Here's the drawing with two shaded views (mm, measured from the low corner). I have some questions. A direction names the side the tool comes from. Give positions to 0.01 mm unless a question says otherwise; leave off trailing zeros. Loops run counter-clockwise (first coordinate to the right, second up) from the corner with the lowest first, then second, coordinate; pieces in that order, holes last. Notation, with made-up numbers: (-18.75, 26) -> (29.25, 26) arc R17 cw to (29.25, 37) -> close; hole circle Ø8 at (57, 52.25). An arc over 180 degrees is marked (long way). Write each question's results on one line, items separated by ' | '. Start each with the question number.
Q1. Which directions (+Z, -Z, +X, -X, +Y, -Y) give clear straight access to the entire face, cutting with the end or side of a thin tool? Please do the marked faces 5, 6 and 7.
Q2. If we section it at D-D, the plane z = 5: List the corners of the cut face in (x, y) for me, plus the area to 3 significant figures.
Q3. If we section it at B-B, the plane z = 23.5: List the corners of the cut face in (x, y) for me.
Q4. If we section it at C-C, the plane y = 7: List the corners of the cut face in (x, z) for me.
Q5. If I drill on line 1 along X through (y, z) = (14, 5); line 2 along X through (y, z) = (1.25, 32); line 3 along X through (y, z) = (7.75, 16), over which ranges is the centre line in solid material (lowest first)?
Q6. Will these pins go through, and if not, where does the flat tip stop? P1, Ø16, axis at x = 81, z = 19.5, coming from the +Y side; P2, Ø5.5, axis at y = 8, z = 22.5, coming from the -X side; P3, Ø1.5, axis at y = 7.5, z = 18, coming from the +X side; P4, Ø2.5, axis at x = 27, z = 5, coming from the -Y side.
Q7. We'd pull the mould along X, two halves only. Please class the marked faces 1, 2, 3 and 4: released by +X, released by -X, zero draft, split by the parting line, or undercut.
Q8. If we section it at A-A, the plane x = 55.5: List the corners of the cut face in (y, z) for me.
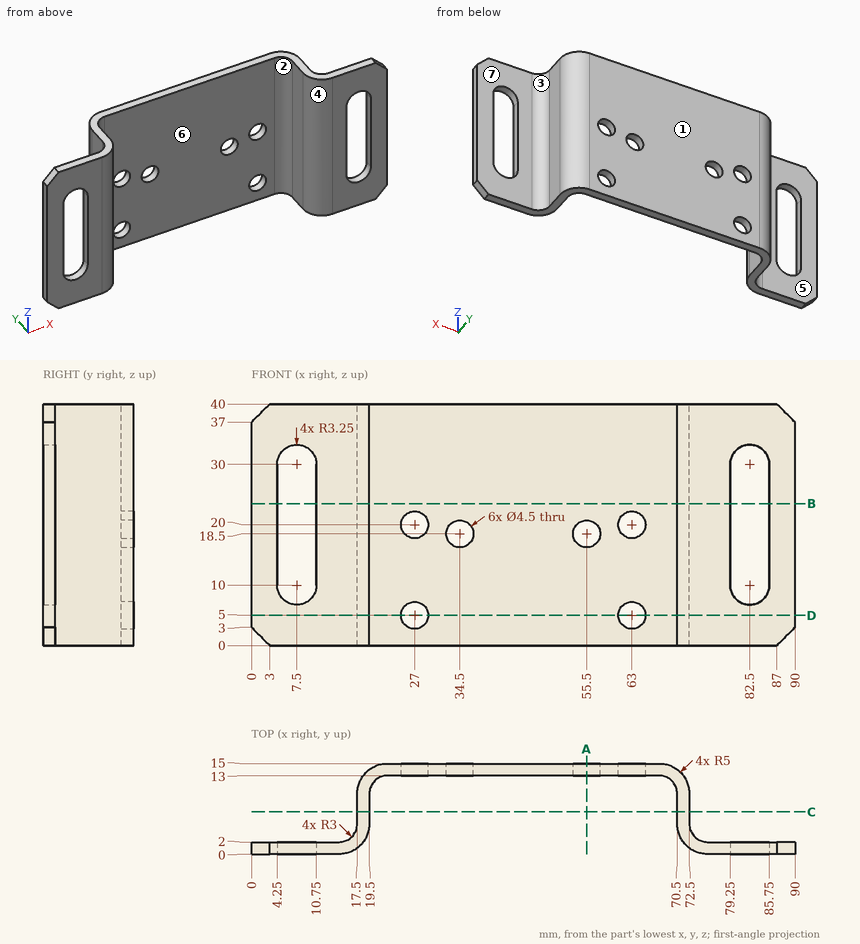
Final values:
1) face 5: +Z, -Z, -X, +Y | face 6: +Z, -Z, -Y | face 7: +Z, -Z, +X, +Y
2) outline: (0, 0) -> (14.5, 0) arc R5 ccw to (19.5, 5) -> (19.5, 10) arc R3 cw to (22.5, 13) -> (24.75, 13) -> (24.75, 15) -> (22.5, 15) arc R5 ccw to (17.5, 10) -> (17.5, 5) arc R3 cw to (14.5, 2) -> (0, 2) -> close; (29.25, 13) -> (60.75, 13) -> (60.75, 15) -> (29.25, 15) -> close; (65.25, 13) -> (67.5, 13) arc R3 cw to (70.5, 10) -> (70.5, 5) arc R5 ccw to (75.5, 0) -> (90, 0) -> (90, 2) -> (75.5, 2) arc R3 cw to (72.5, 5) -> (72.5, 10) arc R5 ccw to (67.5, 15) -> (65.25, 15) -> close | area: 200 mm²
3) outline: (0, 0) -> (4.25, 0) -> (4.25, 2) -> (0, 2) -> close; (10.75, 0) -> (14.5, 0) arc R5 ccw to (19.5, 5) -> (19.5, 10) arc R3 cw to (22.5, 13) -> (67.5, 13) arc R3 cw to (70.5, 10) -> (70.5, 5) arc R5 ccw to (75.5, 0) -> (79.25, 0) -> (79.25, 2) -> (75.5, 2) arc R3 cw to (72.5, 5) -> (72.5, 10) arc R5 ccw to (67.5, 15) -> (22.5, 15) arc R5 ccw to (17.5, 10) -> (17.5, 5) arc R3 cw to (14.5, 2) -> (10.75, 2) -> close; (85.75, 0) -> (90, 0) -> (90, 2) -> (85.75, 2) -> close
4) outline: (17.5, 0) -> (19.5, 0) -> (19.5, 40) -> (17.5, 40) -> close; (70.5, 0) -> (72.5, 0) -> (72.5, 40) -> (70.5, 40) -> close
5) line 1: x = 19.5 to 24.75, 29.25 to 60.75, 65.25 to 70.5 | line 2: x = 0 to 4.94, 10.06 to 17.81, 72.19 to 79.94, 85.06 to 90 | line 3: x = 17.5 to 19.5, 70.5 to 72.5
6) P1: stops at y = 3.34 | P2: stops at x = 17.5 | P3: stops at x = 72.5 | P4: passes through
7) face 1: zero draft | face 2: undercut | face 3: released by +X | face 4: undercut
8) outline: (13, 0) -> (15, 0) -> (15, 16.25) -> (13, 16.25) -> close; (13, 20.75) -> (15, 20.75) -> (15, 40) -> (13, 40) -> close
